from build123d import *

# Parameters (mm, degrees)
SKETCH1_W                                          = 60
SKETCH1_H                                          = 49.5
BOSS_EXTRUDE1_DEPTH                                = 7.5
SKETCH2_W                                          = 26.5
SKETCH2_H                                          = 25
SKETCH2_W_2                                        = 13
SKETCH2_H_2                                        = 8
SKETCH2_W_3                                        = 26
SKETCH2_H_3                                        = 27.5
CUT_EXTRUDE1_DEPTH                                 = 40.60823778
HOLE_WIZARD_SOCKET_HEAD_CAP_SCREW_TYPE_D           = 3.4
HOLE_WIZARD_SOCKET_HEAD_CAP_SCREW_TYPE_CBORE_D     = 6
HOLE_WIZARD_SOCKET_HEAD_CAP_SCREW_TYPE_CBORE_DEPTH = 3.4
F_6_0_6_DIAMETER_HOLE1_D                           = 6
CUT_EXTRUDE2_DEPTH                                 = 1
FILLET1_R                                          = 5
CHAMFER1_SIZE                                      = 10
CHAMFER2_SIZE                                      = 2
FILLET2_R                                          = 3
M4_TAPPED_HOLE1_D                                  = 3.3
SKETCH10_R                                         = 2.75
CUT_EXTRUDE3_DEPTH                                 = 8


with BuildPart() as part:
    # Sketch1 → Boss-Extrude1 (new body)
    with BuildSketch(Plane(origin=(0, 0, 0), x_dir=(1, 0, 0), z_dir=(0, 1, 0))):
        Rectangle(SKETCH1_W, SKETCH1_H)
    extrude(amount=BOSS_EXTRUDE1_DEPTH)

    # Sketch2 → Cut-Extrude1 (cut, through all)
    with BuildSketch(Plane(origin=(0, 7.5, 0), x_dir=(1, 0, 0), z_dir=(0, 1, 0))):
        with Locations((16.75, 12.25)):
            Rectangle(SKETCH2_W, SKETCH2_H)
        with Locations((23.5, -20.75)):
            Rectangle(SKETCH2_W_2, SKETCH2_H_2)
        with Locations((-17, -11)):
            Rectangle(SKETCH2_W_3, SKETCH2_H_3)
    extrude(amount=-CUT_EXTRUDE1_DEPTH, mode=Mode.SUBTRACT)

    # Hole wizard: socket head cap screw, type 1 (through all)
    with Locations(Plane(origin=(0, 7.5, 0), x_dir=(1, 0, 0), z_dir=(0, 1, 0))):
        with Locations((-10.55, 21.25), (-20.55, 21.25), (-20.55, 6.25), (-10.55, 6.25)):
            CounterBoreHole(HOLE_WIZARD_SOCKET_HEAD_CAP_SCREW_TYPE_D / 2, HOLE_WIZARD_SOCKET_HEAD_CAP_SCREW_TYPE_CBORE_D / 2, HOLE_WIZARD_SOCKET_HEAD_CAP_SCREW_TYPE_CBORE_DEPTH)

    # Ø6.0 (6) Diameter Hole1 (through all)
    with Locations(Plane(origin=(0, 7.5, 0), x_dir=(1, 0, 0), z_dir=(0, 1, 0))):
        with Locations((24, -8.5)):
            Hole(F_6_0_6_DIAMETER_HOLE1_D / 2)

    # Sketch7 → Cut-Extrude2 (cut)
    with BuildSketch(Plane(origin=(0, 7.5, 0), x_dir=(1, 0, 0), z_dir=(0, 1, 0))):
        Polygon((-12.304041346, -8.790622211), (20.302775541, -27.616176718), (24.802775541, -19.821948084), (-7.804041346, -0.996393577), align=None)
    extrude(amount=-CUT_EXTRUDE2_DEPTH, mode=Mode.SUBTRACT)

    # Fillet1
    fillet1_edges = [part.edges().sort_by_distance(p)[0] for p in [
        (30, 3.75, 16.75),
        (30, 3.75, 0.25),
    ]]
    fillet(fillet1_edges, radius=FILLET1_R)

    # Chamfer1
    chamfer1_edges = [part.edges().sort_by_distance(p)[0] for p in [
        (3.5, 3.75, -24.75),
    ]]
    chamfer(chamfer1_edges, length=CHAMFER1_SIZE)

    # Chamfer2
    chamfer2_edges = [part.edges().sort_by_distance(p)[0] for p in [
        (17, 3.25, 24.75),
        (-4, 3.75, 24.75),
        (-30, 3.75, -2.75),
        (-30, 3.75, -24.75),
    ]]
    chamfer(chamfer2_edges, length=CHAMFER2_SIZE)

    # Fillet2
    fillet2_edges = [part.edges().sort_by_distance(p)[0] for p in [
        (3.5, 3.75, 0.25),
        (17, 3.25, 16.75),
        (-4, 3.75, -2.75),
    ]]
    fillet(fillet2_edges, radius=FILLET2_R)

    # M4 Tapped Hole1 (through all)
    with Locations(Plane(origin=(0, 7.5, 0), x_dir=(1, 0, 0), z_dir=(0, 1, 0))):
        with Locations((9.538573783, -7.545055475), (2.038573783, -20.535436532)):
            Hole(M4_TAPPED_HOLE1_D / 2)

    # Sketch10 → Cut-Extrude3 (cut)
    with BuildSketch(Plane.ZY.offset(30)):
        with Locations((-13.75, 3.75)):
            Circle(SKETCH10_R)
    extrude(amount=-CUT_EXTRUDE3_DEPTH, mode=Mode.SUBTRACT)


solid = part.part
Part model, mm, in its own coordinate system. A direction names the side the tool comes from. Give positions to 0.01 mm unless a question says otherwise; leave off trailing zeros. Loops run counter-clockwise (first coordinate to the right, second up) from the corner with the lowest first, then second, coordinate; pieces in that order, holes last. Notation, with made-up numbers: M 70.5,3.25 L 74.5,3.25 A13 ccw 74.5,18.25 Z; hole C 3.25,55.25 d4. An arc over 180 degrees is marked long. Put each result on its own line as item: value. Start each with the question number.
1) Saw through at A-A (x = -20.55). List the corners of the cut face in (y, z).
2) Probe probe 1 along Z at (x, y) = (-20.55, 5); probe 2 along Z at (x, y) = (24, 2). List the from-to ranges inside material, lowest first.
3) Saw through at C-C (y = 5.5). State how many separate pieces and enclosed holes the cut face has, then the cut area to 3 significant figures.
4) 3-axis set-ups, long thin cutter, end or side, ignore diameter. For faces 1 (the flat face through (17, 3, 21)), 2 (the flat face through (-22, 4, -14)), 3 (the flat face through (-4, 4, 12)), 4 (the flat face through (-1.57, 3.8, -19.82)), 5 (the cylindrical face through (-7.78, 5.82, -20.1)): which of +Z, -Z, +X, -X, +Y, -Y reach the whole face in a straight line?
5) Saw through at B-B (z = -21.25). List the corners of the cut face in (x, y), then the cut area to 3 significant figures.
6) Flat gauge pins, fed straight in: pin 1 (2.5 mm diameter, centred on x = 2.04, z = 20.54, fed in from -Y); pin 2 (4 mm diameter, centred on x = 9, y = 5.5, fed in from -Z); pin 3 (2 mm diameter, centred on x = -14, y = 5, fed in from +Z); pin 4 (3 mm diameter, centred on x = -21, z = -21, fed in from +Y). Where does each tip first touch, or does it go through?
7) Pull direction X, two halves, no side cores. Call faces 6 (the flat face through (22, 4, 16.75)), 7 (the cylindrical face through (-10.18, 2.02, -4.59)), 8 (the cylindrical face through (8.78, 3.7, 9.01)), 9 (the cylindrical face through (17.9, 3.7, 17.61)): +X half, -X half, draft (parallel to the pull), parting line (faces both ways), or undercut.
8) Saw through at D-D (z = -13.75). List the corners of the cut face in (x, y).
Numbers:
1. outline: M 0,-24.75 L 7.5,-24.75 L 7.5,-24.25 L 4.1,-24.25 L 4.1,-22.95 L 0,-22.95 Z; M 0,-19.55 L 4.1,-19.55 L 4.1,-18.25 L 7.5,-18.25 L 7.5,-9.25 L 4.1,-9.25 L 4.1,-7.95 L 0,-7.95 Z; M 0,-4.55 L 4.1,-4.55 L 4.1,-3.25 L 7.5,-3.25 L 7.5,-2.75 L 0,-2.75 Z
2. probe 1: -24.75 to -24.25, -18.25 to -9.25, -3.25 to -2.75
2. probe 2: 0.25 to 5.5, 11.5 to 16.75
3. separate pieces: 1
3. enclosed holes: 7
3. area: 1,230 mm^2
4. face 1: +Z, +X, +Y, -Y
4. face 2: -X
4. face 3: +Z, -X, +Y, -Y
4. face 4: -Z, +X, +Y, -Y
4. face 5: +Y
5. outline: M -30,0 L -22.25,0 L -22.25,4.1 L -23.55,4.1 L -23.55,7.5 L -30,7.5 Z; M -18.85,0 L -12.25,0 L -12.25,4.1 L -13.55,4.1 L -13.55,7.5 L -17.55,7.5 L -17.55,4.1 L -18.85,4.1 Z; M -8.85,0 L -3,0 L -3,7.5 L -7.55,7.5 L -7.55,4.1 L -8.85,4.1 Z
5. area: 134 mm^2
6. pin 1: through
6. pin 2: z = 0.25
6. pin 3: z = -2.75
6. pin 4: y = 4.1
7. face 6: draft
7. face 7: undercut
7. face 8: undercut
7. face 9: +X half
8. outline: M -30,0 L 3.5,0 L 3.5,7.5 L -30,7.5 L -30,6.5 L -22,6.5 L -22,1 L -30,1 Z
